Geometry: final body of the model. Coordinates: model frame, mm. Face numbers are marked on the shaded views. A direction names the side the tool comes from. Coordinates: 2 decimals unless noted, no trailing zeros. Order: outer loops, then holes, each group sorted by start corner. A loop starts at its lowest first (then second) coordinate and runs counter-clockwise, first axis right, second up. Notation, with made-up numbers: M 86.25,39 L 97.25,39 A21 ccw 97.25,55 Z; hole C 53,8 d6. An arc over 180 degrees is marked long. Use CSV: the item, a comma, the result in double quotes. Start each with the question number.
1. Material intervals for line 1 (Y direction, x = 0.7, z = -30); line 2 (Z direction, x = 2.35, y = -28.5); line 3 (Z direction, x = 2.3, y = -10), sorted ascending.
2. Section query C-C on y = 33. Return the cut outline in (x, z).
3. Section query B-B on y = -9.5. Return the cut outline in (x, z), and give its area (3 significant figures).
4. Section query A-A on z = 0. Return the cut outline in (x, y), and give its area (3 significant figures).
5. Section query D-D on x = 2.1. State how many separate pieces and enclosed holes the cut face has, and give its area (3 significant figures).
6. First-contact query: P1, Ø1.5, axis at y = 17, z = 11.5, coming from the -X side. Flat tip, straight axial feed; report the tip coordinate or a pass-through.
7. Set-up query: the marked faces 1 and 2. Return all of +Z, -Z, +X, -X, +Y, -Y with unobstructed straight access to the full face (end or side cutting, diameter ignored); none if empty.
from build123d import *

# Parameters (mm, degrees)
SKETCH4_R          = 9
CUT_EXTRUDE1_DEPTH = 10


with BuildPart() as part:
    # Sketch2 → Revolve1 (revolve)
    with BuildSketch(Plane.XY):
        with BuildLine():
            Line((6, 0), (6, 18.821530225))
            ThreePointArc((6, 18.821530225), (4.519902914, 19.393505195), (3, 19.849287907))
            Line((3, 19.849287907), (3, 41))
            Line((3, 41), (0, 41))
            Line((0, 41), (0, 0))
            Line((0, 0), (6, 0))
        make_face()
    revolve(axis=Axis((0, 0, 0), (1, 0, 0)))

    # Sketch3 → Cut-Revolve1 (revolve, cut)
    with BuildSketch(Plane.XY, mode=Mode.PRIVATE) as cut_revolve1_sk:
        with BuildLine():
            Line((6, 15.5), (6, 0))
            Line((6, 0), (0, 0))
            Line((0, 0), (0, 17.370620624))
            ThreePointArc((0, 17.370620624), (3.084663444, 16.706867601), (6, 15.5))
        make_face()
    revolve(cut_revolve1_sk.sketch.rotate(Axis((6, 0, 0), (-1, 0, 0)), 270), axis=Axis((6, 0, 0), (-1, 0, 0)), mode=Mode.SUBTRACT)

    # Sketch4 → Cut-Extrude1 (cut)
    with BuildSketch(Plane(origin=(3, 0, 0), x_dir=(0, 0, -1), z_dir=(1, 0, 0))):
        with Locations((0, 29.5)):
            Circle(SKETCH4_R)
        with Locations((18.962234486, 22.598311072)):
            Circle(SKETCH4_R)
        with Locations((29.051828714, 5.122621241)):
            Circle(SKETCH4_R)
        with Locations((25.547749412, -14.75)):
            Circle(SKETCH4_R)
        with Locations((10.089594228, -27.720932313)):
            Circle(SKETCH4_R)
        with Locations((-10.089594228, -27.720932313)):
            Circle(SKETCH4_R)
        with Locations((-25.547749412, -14.75)):
            Circle(SKETCH4_R)
        with Locations((-29.051828714, 5.122621241)):
            Circle(SKETCH4_R)
        with Locations((-18.962234486, 22.598311072)):
            Circle(SKETCH4_R)
    extrude(amount=-CUT_EXTRUDE1_DEPTH, mode=Mode.SUBTRACT)


solid = part.part
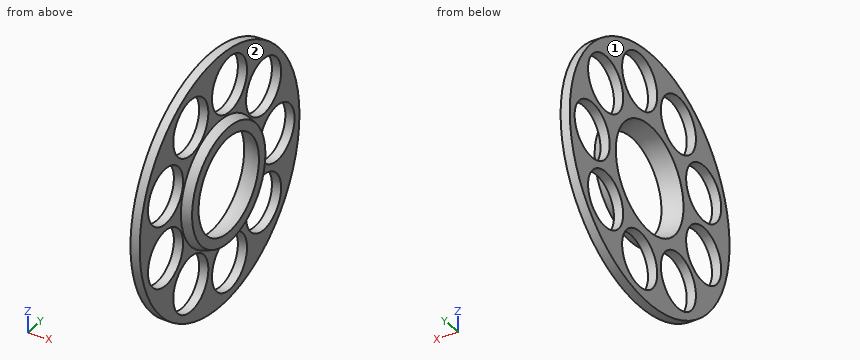
Results list:
1,line 1,"y = -27.95 to -22.57, -6.93 to -3.83, 14.07 to 27.95"
1,line 2,"z = -29.47 to -19.06, -1.12 to 1.12, 19.06 to 29.47"
1,line 3,"z = -39.76 to -33.19, -17.9 to -13.66, 13.66 to 17.9, 33.19 to 39.76"
2,outline,"M 0,-24.33 L 3,-24.33 L 3,-8.29 L 0,-8.29 Z; M 0,8.29 L 3,8.29 L 3,24.33 L 0,24.33 Z"
3,outline,"M 0,-39.88 L 3,-39.88 L 3,-32.86 L 0,-32.86 Z; M 0,-18.24 L 3,-18.24 L 3,-17.43 A18.17 ccw 6,-16.25 L 6,-12.25 A14.7 cw 0,-14.54 Z; M 0,14.54 A14.7 cw 6,12.25 L 6,16.25 A18.17 ccw 3,17.43 L 3,18.24 L 0,18.24 Z; M 0,32.86 L 3,32.86 L 3,39.88 L 0,39.88 Z"
3,area,"89.1 mm²"
4,outline,"M 0,-41 L 3,-41 L 3,-19.85 A20.5 ccw 6,-18.82 L 6,-15.5 A17.5 cw 0,-17.37 Z; M 0,17.37 A17.5 cw 6,15.5 L 6,18.82 A20.5 ccw 3,19.85 L 3,20.5 L 0,20.5 Z; M 0,38.5 L 3,38.5 L 3,41 L 0,41 Z"
4,area,"109 mm²"
5,separate pieces,"1"
5,enclosed holes,"10"
5,area,"2,080 mm²"
6,P1,"stops at x = 0"
7,face 1,"+Z, -Z, -X, +Y, -Y"
7,face 2,"+X"
